The model under review builds one solid part; all positions refer to its coordinate system, in mm. Face numbers are marked on the shaded views. A direction names the side the tool comes from. Give positions to 0.01 mm unless a question says otherwise; leave off trailing zeros. Order: outer loops, then holes, each group sorted by start corner. A loop starts at its lowest first (then second) coordinate and runs counter-clockwise, first axis right, second up. Notation, with made-up numbers: (68.5, 53.25) - (83.5, 53.25) arc R31 ccw to (83.5, 77.25) - close; hole circle Ø9 at (50.5, -7). An arc over 180 degrees is marked (long way). Put each result on its own line as item: value.
```python
from build123d import *

# Parameters (mm, degrees)
SKETCH1_W           = 42
SKETCH1_H           = 42
SKETCH1_R           = 1.5
BOSS_EXTRUDE1_DEPTH = 47
CUT_EXTRUDE1_DEPTH  = 56.596762496
SKETCH4_R           = 11
BOSS_EXTRUDE2_DEPTH = 2
BOSS_EXTRUDE3_DEPTH = 40
CUT_EXTRUDE2_DEPTH  = 2
SKETCH8_R           = 3
CUT_EXTRUDE3_DEPTH  = 2
BOSS_EXTRUDE4_START = 1.9
SKETCH9_R           = 2.5
BOSS_EXTRUDE4_DEPTH = 1.9
SKETCH10_W          = 3
SKETCH10_H          = 10.31009041
SKETCH10_W_2        = 2.478607588
SKETCH10_H_2        = 8.518222776
BOSS_EXTRUDE5_DEPTH = 5
SKETCH11_R          = 0.5
BOSS_EXTRUDE6_DEPTH = 5


with BuildPart() as part:
    # Sketch1 → Boss-Extrude1 (new body)
    with BuildSketch(Plane.XY):
        Rectangle(SKETCH1_W, SKETCH1_H)
        with Locations((-15.5, 15.5)):
            Circle(SKETCH1_R, mode=Mode.SUBTRACT)
        with Locations(Location((15.5, 15.5, 0), (0, 0, 180))):
            Circle(SKETCH1_R, mode=Mode.SUBTRACT)
        with Locations(Location((-15.5, -15.5, 0), (0, 0, 180))):
            Circle(SKETCH1_R, mode=Mode.SUBTRACT)
        with Locations((15.5, -15.5)):
            Circle(SKETCH1_R, mode=Mode.SUBTRACT)
    extrude(amount=BOSS_EXTRUDE1_DEPTH)

    # Sketch3 → Cut-Extrude1 (cut, through all)
    with BuildSketch(Plane(origin=(0, 0, 0), x_dir=(-1, 0, 0), z_dir=(0, 0, -1))):
        Polygon((-21, 17), (-17, 21), (-21, 21), align=None)
        Polygon((21, 21), (17, 21), (21, 17), align=None)
        Polygon((21, -17), (17, -21), (21, -21), align=None)
        Polygon((-21, -21), (-17, -21), (-21, -17), align=None)
    extrude(amount=-CUT_EXTRUDE1_DEPTH, mode=Mode.SUBTRACT)

    # Sketch4 → Boss-Extrude2 (add)
    with BuildSketch(Plane(origin=(0, 0, 0), x_dir=(-1, 0, 0), z_dir=(0, 0, -1))):
        Circle(SKETCH4_R)
    extrude(amount=BOSS_EXTRUDE2_DEPTH)

    # Sketch5 → Boss-Extrude3 (add)
    with BuildSketch(Plane(origin=(0, 0, -2), x_dir=(-1, 0, 0), z_dir=(0, 0, -1))):
        with BuildLine():
            Line((1.7, -1.833030278), (1.7, 1.833030278))
            ThreePointArc((1.7, 1.833030278), (-2.5, 0), (1.7, -1.833030278))
        make_face()
    extrude(amount=BOSS_EXTRUDE3_DEPTH)

    # Sketch7 → Cut-Extrude2 (cut)
    with BuildSketch(Plane.XY.offset(47)):
        with BuildLine():
            Line((21, 17), (21, 11.625484678))
            ThreePointArc((21, 11.625484678), (13.597062084, 13.597062084), (11.625484678, 21))
            Line((11.625484678, 21), (17, 21))
            Line((17, 21), (21, 17))
        make_face()
        with BuildLine():
            Line((-21, -17), (-21, -11.625484678))
            ThreePointArc((-21, -11.625484678), (-13.597062084, -13.597062084), (-11.625484678, -21))
            Line((-11.625484678, -21), (-17, -21))
            Line((-17, -21), (-21, -17))
        make_face()
        with BuildLine():
            Line((-11.625484678, 21), (-17, 21))
            Line((-17, 21), (-21, 17))
            Line((-21, 17), (-21, 11.625484678))
            ThreePointArc((-21, 11.625484678), (-13.597062084, 13.597062084), (-11.625484678, 21))
        make_face()
        with BuildLine():
            Line((11.625484678, -21), (17, -21))
            Line((17, -21), (21, -17))
            Line((21, -17), (21, -11.625484678))
            ThreePointArc((21, -11.625484678), (13.597062084, -13.597062084), (11.625484678, -21))
        make_face()
    extrude(amount=-CUT_EXTRUDE2_DEPTH, mode=Mode.SUBTRACT)

    # Sketch8 → Cut-Extrude3 (cut)
    with BuildSketch(Plane.XY.offset(47)):
        Circle(SKETCH8_R)
    extrude(amount=-CUT_EXTRUDE3_DEPTH, mode=Mode.SUBTRACT)

    # Sketch9 → Boss-Extrude4 (add)
    with BuildSketch(Plane.XY.offset(45).offset(BOSS_EXTRUDE4_START)):
        with Locations(Location((0, 0, 0), (0, 0, 180))):
            Circle(SKETCH9_R)
    extrude(amount=-BOSS_EXTRUDE4_DEPTH)

    # Sketch10 → Boss-Extrude5 (add)
    with BuildSketch(Plane.ZY.offset(21)):
        with Locations((45.5, 0)):
            Rectangle(SKETCH10_W, SKETCH10_H)
        with Locations((45.5, 0)):
            Rectangle(SKETCH10_W_2, SKETCH10_H_2, mode=Mode.SUBTRACT)
    extrude(amount=BOSS_EXTRUDE5_DEPTH)

    # Sketch11 → Boss-Extrude6 (add)
    with BuildSketch(Plane.ZY.offset(21)):
        with Locations(Location((45.5, 3.127782029, 0), (0, 0, 180))):
            Circle(SKETCH11_R)
        with Locations(Location((45.5, 1.627782029, 0), (0, 0, 180))):
            Circle(SKETCH11_R)
        with Locations(Location((45.5, 0.127782029, 0), (0, 0, 180))):
            Circle(SKETCH11_R)
        with Locations(Location((45.5, -1.372217971, 0), (0, 0, 180))):
            Circle(SKETCH11_R)
        with Locations(Location((45.5, -2.872217971, 0), (0, 0, 180))):
            Circle(SKETCH11_R)
    extrude(amount=BOSS_EXTRUDE6_DEPTH)


solid = part.part
```
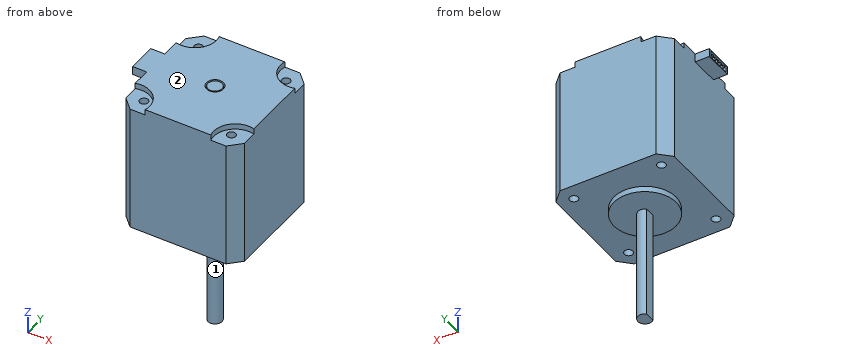
(1) Wall thickness on L1, parallel to X at y = 15.5, z = 32; L2, parallel to Y at x = -16, z = 40: over which ranges is each line inside the solid? List them lowest first.
The answers:
L1: -21 to -17, -14 to 14, 17 to 21
L2: -21 to -16.91, -14.09 to 14.09, 16.91 to 21
(2) Take a section at B-B, the plane z = 19.5. Write out the cut boundary in (x, y), then the cut area to 3 significant figures.
The answers:
outline: (-21, -17) - (-17, -21) - (17, -21) - (21, -17) - (21, 17) - (17, 21) - (-17, 21) - (-21, 17) - close; hole circle Ø3 at (-15.5, -15.5); hole circle Ø3 at (-15.5, 15.5); hole circle Ø3 at (15.5, -15.5); hole circle Ø3 at (15.5, 15.5)
area: 1,700 mm^2
(3) Clearance check with flat-ended pins moving along their axes: pin 1 Ø1.2 at (x, z) = (-23.5, 45.5) entering from -Y; pin 2 Ø7.5 at (x, y) = (-17.5, -16.5) entering from +Z; pin 3 Ø1.1 at (y, z) = (1, -30.5) entering from -X. State where each tip first meets the part, or that it passes through.
The answers:
pin 1: y = -5.16
pin 2: z = 45
pin 3: x = -1.7
(4) For the marked faces 1 and 2, list the 3-axis set-ups (+Z, -Z, +X, -X, +Y, -Y) from which the entire face can be reached by the end or side of a thin tool; tool diameter is ignored.
The answers:
face 1: -Z
face 2: +Z, +X, -X, +Y, -Y
(5) Take a section at A-A, the plane y = 15.5. Write out the cut boundary in (x, z).
The answers:
outline: (-21, 0) - (-17, 0) - (-17, 45) - (-21, 45) - close; (-14, 0) - (14, 0) - (14, 45) - (12.21, 45) - (12.21, 47) - (-12.21, 47) - (-12.21, 45) - (-14, 45) - close; (17, 0) - (21, 0) - (21, 45) - (17, 45) - close
(6) Take a section at C-C, the plane x = 0. Write out the cut boundary in (y, z), then the cut area to 3 significant figures.
The answers:
outline: (-21, 0) - (-11, 0) - (-11, -2) - (-2.5, -2) - (-2.5, -42) - (2.5, -42) - (2.5, -2) - (11, -2) - (11, 0) - (21, 0) - (21, 47) - (3, 47) - (3, 45) - (2.5, 45) - (2.5, 46.9) - (-2.5, 46.9) - (-2.5, 45) - (-3, 45) - (-3, 47) - (-21, 47) - close
area: 2,220 mm^2
